Verification items for the finished model (mm, model axes). A direction names the side the tool comes from. Round coordinates to 2 decimals unless told otherwise and drop trailing zeros. Loops run counter-clockwise (first coordinate to the right, second up) from the corner with the lowest first, then second, coordinate; pieces in that order, holes last. Notation, with made-up numbers: (-25.75, 48.5) -> (4.25, 48.5) arc R29 ccw to (4.25, 72.5) -> close; hole circle Ø7 at (54.5, 18). An arc over 180 degrees is marked (long way). Write item = value, one per line.
```python
from build123d import *

# Parameters (mm, degrees)
BASE_BLOCK_SKETCH_W = 48
BASE_BLOCK_SKETCH_H = 48
BASE_BLOCK_DEPTH    = 28
HOOK_ARM_DEPTH      = 48
EYE_ARM_DEPTH       = 48
EYE_BOSS_DEPTH      = 20
EYE_BORE_SKETCH_R   = 16.5
EYE_BORE_33_DEPTH   = 20
HOOK_END_DEPTH      = 20
HOOK_SLOT_32_DEPTH  = 20


with BuildPart() as part:
    # Base Block Sketch → Base Block (new body)
    with BuildSketch(Plane.XY):
        with Locations((24, -24)):
            Rectangle(BASE_BLOCK_SKETCH_W, BASE_BLOCK_SKETCH_H)
    extrude(amount=BASE_BLOCK_DEPTH)

    # Hook Arm Sketch → Hook Arm (add)
    with BuildSketch(Plane(origin=(0, 0, 0), x_dir=(1, 0, 0), z_dir=(0, 1, 0))):
        Polygon((34, -28), (24, -28), (14, -28), (14, -48), (34, -48), align=None)
    extrude(amount=-HOOK_ARM_DEPTH)

    # Eye Arm Sketch → Eye Arm (add)
    with BuildSketch(Plane(origin=(48, 0, 0), x_dir=(0, 0, -1), z_dir=(1, 0, 0))):
        Polygon((0, -24), (0, -14), (20, -14), (20, -34), (0, -34), align=None)
    extrude(amount=-EYE_ARM_DEPTH)

    # Eye Boss Sketch → Eye Boss (add)
    with BuildSketch(Plane(origin=(0, -14, 0), x_dir=(1, 0, 0), z_dir=(0, 1, 0))):
        with BuildLine():
            Line((0, 20), (48, 20))
            ThreePointArc((48, 20), (24, 44), (0, 20))
        make_face()
    extrude(amount=-EYE_BOSS_DEPTH)

    # Eye Bore Sketch → Eye Bore Ø33 (cut)
    with BuildSketch(Plane(origin=(0, -14, 0), x_dir=(1, 0, 0), z_dir=(0, 1, 0))):
        with Locations(Location((24, 20, 0), (0, 0, 270))):
            Circle(EYE_BORE_SKETCH_R)
    extrude(amount=-EYE_BORE_33_DEPTH, mode=Mode.SUBTRACT)

    # Hook End Sketch → Hook End (add)
    with BuildSketch(Plane(origin=(34, 0, 0), x_dir=(0, 0, -1), z_dir=(1, 0, 0))):
        with BuildLine():
            Line((-67.598850506, -8.002873735), (-48, -8.002873735))
            Line((-48, -8.002873735), (-48, 0))
            ThreePointArc((-48, 0), (-58.584905871, -2.077813215), (-67.598850506, -8.002873735))
        make_face()
        with BuildLine():
            Line((-48, -48), (-48, -39.997126265))
            Line((-48, -39.997126265), (-68, -39.997126265))
            ThreePointArc((-68, -39.997126265), (-58.800418806, -45.998891596), (-48, -48))
        make_face()
    extrude(amount=-HOOK_END_DEPTH)

    # Hook Slot Sketch → Hook Slot 32 (cut)
    with BuildSketch(Plane(origin=(34, 0, 0), x_dir=(0, 0, -1), z_dir=(1, 0, 0))):
        with BuildLine():
            Line((-48, -8), (-48, -8.002873735))
            Line((-48, -8.002873735), (-48, -39.997126265))
            Line((-48, -39.997126265), (-48, -40))
            ThreePointArc((-48, -40), (-32, -24), (-48, -8))
        make_face()
    extrude(amount=-HOOK_SLOT_32_DEPTH, mode=Mode.SUBTRACT)


solid = part.part
```
(1) Draft check along X on faces 1 (the face through (34, -13, 35)), 2 (the face through (17.68, -23.86, -4.76)), 3 (the face through (24, 0, 18)). Enter one of: released by +X, released by -X, zero draft, split by the parting line, or undercut.
Filled sheet:
face_1 = released by +X
face_2 = undercut
face_3 = zero draft
(2) Go/stop test with flat-tipped pins: pin 1 Ø12 at (y, z) = (-13, 43) entering from +X; pin 2 Ø8 at (y, z) = (-13, -28) entering from -X; pin 3 Ø15.5 at (x, z) = (28.5, 62.5) entering from -Y. Record where each tip stops, or that it passes through.
Filled sheet:
pin_1 = 34
pin_2 = 0.36
pin_3 = -47.27
(3) Set-up check for faces 4 (the face through (8, -34, -13)), 5 (the face through (24, -8.003, 58)), 6 (the face through (8, -14, -13)): record each of +Z, -Z, +X, -X, +Y, -Y from which the full face is reachable in a straight line by a thin tool's end or side.
Filled sheet:
face_4 = -Z, +X, -X, -Y
face_5 = +Z, +X, -X
face_6 = -Z, +X, -X, +Y
(4) Sectioned sample at C-C, the plane z = -26. Record the cut outline in (x, y).
Filled sheet:
outline = (0.76, -34) -> (8.63, -34) -> (8.63, -14) -> (0.76, -14) -> close; (39.37, -34) -> (47.24, -34) -> (47.24, -14) -> (39.37, -14) -> close
(5) Sectioned sample at D-D, the plane z = 60. Record the cut outline in (x, y), and give its area (3 significant figures).
Filled sheet:
outline = (14, -45.49) -> (34, -45.49) -> (34, -40) -> (14, -40) -> close; (14, -8) -> (34, -8) -> (34, -2.7) -> (14, -2.7) -> close
area = 216 mm2
(6) Material ranges on probe 1 along X at (y, z) = (-29, -20); probe 2 along Z at (x, y) = (38, -37); probe 3 along Y at (x, z) = (19, 5.5), recorded low to high. Write a range as from..to.
Filled sheet:
probe_1 = 0..7.5, 40.5..48
probe_2 = 0..28
probe_3 = -48..0
(7) Sectioned sample at B-B, the plane y = -24. Record the cut outline in (x, z), and give its area (3 significant figures).
Filled sheet:
outline = (0, -20) arc R24 ccw to (48, -20) -> (48, 28) -> (34, 28) -> (34, 32) -> (14, 32) -> (14, 28) -> (0, 28) -> close; hole circle Ø33 at (24, -20)
area = 2,430 mm2
